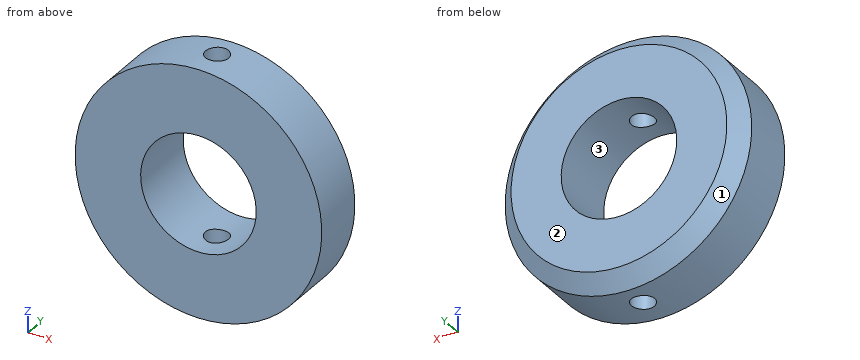
from build123d import *

# Parameters (mm, degrees)
COLLAR_RING_PROFILE_R   = 16
COLLAR_RING_PROFILE_R_2 = 7.5
COLLAR_BODY_DEPTH       = 9
EDGE_CHAMFER_2X45_SIZE  = 2
CROSS_HOLE_3_DEPTH      = 25.351591324
CROSS_HOLE_3_DEPTH_BACK = 25.351591324
CROSS_HOLE_PROFILE_R    = 1.5


with BuildPart() as part:
    # Collar Ring Profile → Collar Body (new body)
    with BuildSketch(Plane(origin=(0, 0, 0), x_dir=(1, 0, 0), z_dir=(0, 1, 0))):
        with Locations(Location((0, 0, 0), (0, 0, 270))):
            Circle(COLLAR_RING_PROFILE_R)
        with Locations(Location((0, 0, 0), (0, 0, 270))):
            Circle(COLLAR_RING_PROFILE_R_2, mode=Mode.SUBTRACT)
    extrude(amount=COLLAR_BODY_DEPTH)

    # Edge Chamfer 2x45
    edge_chamfer_2x45_edges = [part.edges().sort_by_distance(p)[0] for p in [
        (0, 9, -16),
    ]]
    chamfer(edge_chamfer_2x45_edges, length=EDGE_CHAMFER_2X45_SIZE)

    # Cross Hole Profile → Cross Hole Ø3 (cut, two sides: drawn at the far end of the back side and taken through both)
    with BuildSketch(Plane.XY.offset(-CROSS_HOLE_3_DEPTH_BACK)):
        with Locations((0, 3.930345363)):
            Circle(CROSS_HOLE_PROFILE_R)
    extrude(amount=CROSS_HOLE_3_DEPTH + CROSS_HOLE_3_DEPTH_BACK, mode=Mode.SUBTRACT)


solid = part.part
Read the model definition and answer for the solid it produces. Units are mm, in the model's axes. Face numbers are marked on the shaded views. Round coordinates to 2 decimals unless told otherwise and drop trailing zeros. Order: outer loops, then holes, each group sorted by start corner. A loop starts at its lowest first (then second) coordinate and runs counter-clockwise, first axis right, second up.
1) Flat-ended cylindrical pins translate along their axes: pin 1 (5 mm diameter, centred on x = 3.5, y = 2, fed in from -Z); pin 2 (1.5 mm diameter, centred on y = 5, z = -10, fed in from +X); pin 3 (1.5 mm diameter, centred on x = 11, y = 8, fed in from +Z). Find the tip coordinate at first contact, or state that the pin passes through.
2) The part is cut by section D-D on y = 2. Write down the section's boundary in (x, z), plus the area to 3 significant figures.
3) The part is cut by section C-C on y = 8.5. Write down the section's boundary in (x, z), plus the area to 3 significant figures.
4) Straight lines are drawn through the part: L1, parallel to X at y = 4.5, z = 0; L2, parallel to X at y = 3.5, z = -10.5; L3, parallel to Z at x = 2, y = 5.5. For each, find the intervals that lie inside material, in ascending order.
5) The part is cut by section A-A on x = 0. Write down the section's boundary in (y, z), plus the area to 3 significant figures.
6) The mould has two halves that part along Z. Classify the marked faces 1, 2 and 3: released by +Z, released by -Z, zero draft, split by the parting line, or undercut.
7) The part is cut by section B-B on z = 0. Write down the section's boundary in (x, y), plus the area to 3 significant figures.
Resolved:
1. pin 1: stops at z = -15.97
1. pin 2: stops at x = 13.06
1. pin 3: stops at z = 11.49
2. outline: circle Ø32 at (0, 0); hole circle Ø15 at (0, 0)
2. area: 628 mm2
3. outline: circle Ø29 at (0, 0); hole circle Ø15 at (0, 0)
3. area: 484 mm2
4. L1: x = -16 to -7.5, 7.5 to 16
4. L2: x = -12.07 to -1.44, 1.44 to 12.07
4. L3: z = -15.87 to -7.23, 7.23 to 15.87
5. outline: (0, -16) - (2.43, -16) - (2.43, -7.5) - (0, -7.5) - close; (0, 7.5) - (2.43, 7.5) - (2.43, 16) - (0, 16) - close; (5.43, -16) - (7, -16) - (9, -14) - (9, -7.5) - (5.43, -7.5) - close; (5.43, 7.5) - (9, 7.5) - (9, 14) - (7, 16) - (5.43, 16) - close
5. area: 98.0 mm2
6. face 1: split by the parting line
6. face 2: zero draft
6. face 3: undercut
7. outline: (-16, 0) - (-7.5, 0) - (-7.5, 9) - (-14, 9) - (-16, 7) - close; (7.5, 0) - (16, 0) - (16, 7) - (14, 9) - (7.5, 9) - close
7. area: 149 mm2
